```python
from build123d import *

# Parameters (mm, degrees)
BOSS_EXTRUDE1_DEPTH     = 680
CUT_EXTRUDE1_DEPTH      = 683.126088051
CUT_EXTRUDE1_DEPTH_BACK = 683.126088051
SKETCH3_R               = 6.5
CUT_EXTRUDE2_DEPTH      = 10


with BuildPart() as part:
    # Sketch1 → Boss-Extrude1 (new body)
    with BuildSketch(Plane.XY):
        with BuildLine():
            Line((0, 40), (0, 0))
            Line((0, 0), (40, 0))
            Line((40, 0), (40, 2))
            ThreePointArc((40, 2), (39.414213562, 3.414213562), (38, 4))
            Line((38, 4), (8, 4))
            ThreePointArc((8, 4), (5.171572875, 5.171572875), (4, 8))
            Line((4, 8), (4, 38))
            ThreePointArc((4, 38), (3.414213562, 39.414213562), (2, 40))
            Line((2, 40), (0, 40))
        make_face()
    extrude(amount=BOSS_EXTRUDE1_DEPTH)

    # Sketch2 → Cut-Extrude1 (cut, two sides: drawn at the far end of the back side and taken through both)
    with BuildSketch(Plane(origin=(0, 4, 0), x_dir=(1, 0, 0), z_dir=(0, 1, 0)).offset(-CUT_EXTRUDE1_DEPTH_BACK)):
        Polygon((0, 0), (40, -40), (40, 0), align=None)
        Polygon((0, -680), (40, -680), (40, -640), align=None)
    extrude(amount=CUT_EXTRUDE1_DEPTH + CUT_EXTRUDE1_DEPTH_BACK, mode=Mode.SUBTRACT)

    # Sketch3 → Cut-Extrude2 (cut)
    with BuildSketch(Plane(origin=(0, 4, 0), x_dir=(1, 0, 0), z_dir=(0, 1, 0))):
        with Locations(Location((25, -140, 0), (0, 0, 180))):
            Circle(SKETCH3_R)
        with Locations(Location((25, -340, 0), (0, 0, 180))):
            Circle(SKETCH3_R)
        with Locations(Location((25, -540, 0), (0, 0, 180))):
            Circle(SKETCH3_R)
    extrude(amount=-CUT_EXTRUDE2_DEPTH, mode=Mode.SUBTRACT)


solid = part.part
```
Can you work these out from the model? Positions are in its coordinate system, mm. A direction names the side the tool comes from. Coordinates: 2 decimals unless noted, no trailing zeros. Order: outer loops, then holes, each group sorted by start corner. A loop starts at its lowest first (then second) coordinate and runs counter-clockwise, first axis right, second up. Notation, with made-up numbers: (23, -27.5) -> (80, -27.5) arc R22 ccw to (80, 9.5) -> close; hole circle Ø7 at (7.5, -21.5). An arc over 180 degrees is marked (long way). Write each question's results on one line, items separated by ' | '.
Item 1: I want a section at A-A, the plane x = 25. Write out the boundary of the cut face in (y, z), then the cut area to 3 significant figures.
Results are:
outline: (0, 25) -> (4, 25) -> (4, 133.5) -> (0, 133.5) -> close; (0, 146.5) -> (4, 146.5) -> (4, 333.5) -> (0, 333.5) -> close; (0, 346.5) -> (4, 346.5) -> (4, 533.5) -> (0, 533.5) -> close; (0, 546.5) -> (4, 546.5) -> (4, 655) -> (0, 655) -> close | area: 2,360 mm²
Item 2: Which directions (+Z, -Z, +X, -X, +Y, -Y) give clear straight access to the entire face, cutting with the end or side of a thin tool? Please do faces 1 (the face through (30.158, 2.028, 136.045)), 2 (the face through (20, 4, 335)).
Results are:
face 1: +Y, -Y | face 2: +Z, -Z, +X, +Y
Item 3: If I drill on line 1 along X through (y, z) = (1, 340); line 2 along Z through (x, y) = (25, 2); line 3 along X through (y, z) = (16, 651.5), over which ranges is the centre line in solid material (lowest first)?
Results are:
line 1: 0 to 18.5, 31.5 to 40 | line 2: 25 to 133.5, 146.5 to 333.5, 346.5 to 533.5, 546.5 to 655 | line 3: 0 to 4
Item 4: If we mould it in two halves opening along X, with no side actions, what happens to faces 3 (the face through (21.506, 2.028, 345.481)), 4 (the face through (0, 20, 335)), 5 (the face through (4, 23, 335))? For each: +X half, -X half, draft (parallel to the pull), parting line (faces both ways), or undercut.
Results are:
face 3: undercut | face 4: -X half | face 5: +X half
Item 5: I want a section at B-B, the plane z = 140. Write out the boundary of the cut face in (x, y).
Results are:
outline: (0, 0) -> (18.5, 0) -> (18.5, 4) -> (8, 4) arc R4 cw to (4, 8) -> (4, 38) arc R2 ccw to (2, 40) -> (0, 40) -> close; (31.5, 0) -> (40, 0) -> (40, 2) arc R2 ccw to (38, 4) -> (31.5, 4) -> close
Item 6: I'm going to push flat-ended pins straight in: pin 1 Ø8 at (y, z) = (33.5, 392) entering from +X; pin 2 Ø10.5 at (x, z) = (25, 340) entering from +Y; pin 3 Ø1 at (x, z) = (35.5, 529.5) entering from +Y. Where does each tip first touch, or does it pass through?
Results are:
pin 1: x = 4 | pin 2: through | pin 3: y = 4
